Model file for the job. Use its own axes, mm. A direction names the side the tool comes from. Round coordinates to 2 decimals unless told otherwise and drop trailing zeros. Write each loop counter-clockwise with the first axis right and the second up, starting at its lowest first coordinate (ties: lowest second). Pieces come first, ordered by that corner, then holes. Notation, with made-up numbers: (9, 56) - (60, 56) arc R23 ccw to (60, 90) - close; hole circle Ø6 at (16.25, 84). An arc over 180 degrees is marked (long way). Answer as a JSON object with one key per item and string values. Group by question number.
from build123d import *

# Parameters (mm, degrees)
BOSS_EXTRUDE_1_DEPTH   = 4
BOSS_EXTRUDE_2_DEPTH   = 4
FILLET_1_R             = 5
SKETCH_6_W             = 24
SKETCH_6_H             = 30
BOSS_EXTRUDE_3_DEPTH   = 3.5
SKETCH_3_R             = 2.25
CUT_EXTRUDE_1_DEPTH    = 191.738695602
LINEAR_PATTERN_1_COUNT = 3
LINEAR_PATTERN_1_PITCH = 10
SKETCH_7_W             = 63.778369094
SKETCH_7_H             = 56.242484603
CUT_EXTRUDE_2_DEPTH    = 10
CHAMFER_3_SIZE         = 1
SKETCH_8_W             = 4.5
SKETCH_8_H             = 30
BOSS_EXTRUDE_4_DEPTH   = 3.5
CUT_EXTRUDE_START      = -10
CUT_EXTRUDE_3_DEPTH    = 10
F_4_0_4_HOLE_1_D       = 4
LINEAR_PATTERN_2_COUNT = 2
LINEAR_PATTERN_2_PITCH = 20


with BuildPart() as part:
    # Sketch 1 → Boss-Extrude 1 (new body)
    with BuildSketch(Plane.XZ.offset(2)):
        with BuildLine():
            Line((-59, 15), (-69, 15))
            Line((-69, 15), (-70, 15))
            Line((-70, 15), (-70, -15))
            Line((-70, -15), (-69, -15))
            Line((-69, -15), (69, -15))
            Line((69, -15), (70, -14))
            Line((70, -14), (70, -1))
            Line((70, -1), (69, 0))
            Line((69, 0), (-53, 0))
            ThreePointArc((-53, 0), (-56.535533906, 1.464466094), (-58, 5))
            Line((-58, 5), (-58, 15))
            Line((-58, 15), (-59, 15))
        make_face()
    extrude(amount=-BOSS_EXTRUDE_1_DEPTH)

    # Sketch 2 → Boss-Extrude 2 (add)
    with BuildSketch(Plane(origin=(0, 2, 0), x_dir=(1, 0, 0), z_dir=(0, 1, 0))):
        Polygon((-70, 15), (-190, 15), (-190, 0), (-82, 0), (-82, -15), (-70, -15), align=None)
    extrude(amount=-BOSS_EXTRUDE_2_DEPTH)

    # Fillet 1
    fillet_1_edges = [part.edges().sort_by_distance(p)[0] for p in [
        (-82, 0, 0),
    ]]
    fillet(fillet_1_edges, radius=FILLET_1_R)

    # Sketch 6 → Boss-Extrude 3 (add)
    with BuildSketch(Plane.XZ.offset(2)):
        with Locations((-70, 0)):
            Rectangle(SKETCH_6_W, SKETCH_6_H)
    extrude(amount=BOSS_EXTRUDE_3_DEPTH)

    # Sketch 3 → Cut-Extrude 1 (cut, through all)
    with BuildSketch(Plane(origin=(0, 2, 0), x_dir=(1, 0, 0), z_dir=(0, 1, 0))):
        with Locations(Location((-70, -10, 0), (0, 0, 270))):
            Circle(SKETCH_3_R)
    cut_extrude_1 = extrude(amount=-CUT_EXTRUDE_1_DEPTH, mode=Mode.SUBTRACT)

    # Linear Pattern 1: Cut-Extrude 1 ×3
    with Locations(*[(0, 0, -i * LINEAR_PATTERN_1_PITCH) for i in range(1, LINEAR_PATTERN_1_COUNT)]):
        add(cut_extrude_1, mode=Mode.SUBTRACT)

    # Sketch 7 → Cut-Extrude 2 (cut)
    with BuildSketch(Plane(origin=(0, 2, 0), x_dir=(1, 0, 0), z_dir=(0, 1, 0))):
        with Locations((81.889184547, 6.971733155)):
            Rectangle(SKETCH_7_W, SKETCH_7_H)
    extrude(amount=-CUT_EXTRUDE_2_DEPTH, mode=Mode.SUBTRACT)

    # Chamfer 3
    chamfer_3_edges = [part.edges().sort_by_distance(p)[0] for p in [
        (50, 0, -15),
        (50, 0, 0),
        (-190, 0, -15),
        (-190, 0, 0),
    ]]
    chamfer(chamfer_3_edges, length=CHAMFER_3_SIZE)

    # Sketch 8 → Boss-Extrude 4 (add)
    with BuildSketch(Plane.XZ.offset(5.5)):
        with Locations((-55.75, 0)):
            Rectangle(SKETCH_8_W, SKETCH_8_H)
        with Locations((-84.25, 0)):
            Rectangle(SKETCH_8_W, SKETCH_8_H)
    extrude(amount=-BOSS_EXTRUDE_4_DEPTH)

    # Sketch 9 → Cut-Extrude 3 (cut)
    with BuildSketch(Plane(origin=(0, -2, 0), x_dir=(1, 0, 0), z_dir=(0, 1, 0)).offset(CUT_EXTRUDE_START)):
        with BuildLine():
            Line((-53.5, -15), (-58, -15))
            Line((-58, -15), (-58, -5))
            ThreePointArc((-58, -5), (-56.708099244, -1.645898034), (-53.5, -0.025062814))
            Line((-53.5, -0.025062814), (-53.5, -15))
        make_face()
        with BuildLine():
            Line((-82, -15), (-86.5, -15))
            Line((-86.5, -15), (-86.5, -0.025062814))
            ThreePointArc((-86.5, -0.025062814), (-83.291900756, -1.645898034), (-82, -5))
            Line((-82, -5), (-82, -15))
        make_face()
    extrude(amount=CUT_EXTRUDE_3_DEPTH, mode=Mode.SUBTRACT)

    # Ø4.0 (4) Hole 1 (through all)
    with Locations(Plane(origin=(0, 2, 0), x_dir=(-1, 0, 0), z_dir=(0, 1, 0))):
        with Locations((60, -7.5)):
            f_4_0_4_hole_1 = Hole(F_4_0_4_HOLE_1_D / 2)

    # Linear Pattern 2: Ø4.0 (4) Hole 1 ×2
    with Locations(*[(-i * LINEAR_PATTERN_2_PITCH, 0, 0) for i in range(1, LINEAR_PATTERN_2_COUNT)]):
        add(f_4_0_4_hole_1, mode=Mode.SUBTRACT)


solid = part.part
(1) Slice it at D-D (x = -31). Write the cut outline in (y, z).
(2) Slice it at C-C (z = 10). Write the cut outline in (x, y).
(3) Drill centre lines: line 1 (X direction, y = -1.5, z = 10); line 2 (Z direction, x = -60, y = -3.5); line 3 (X direction, y = -4, z = -10). Where is each one in solid material? Low to high. Write a range as from..to.
(4) Slice it at A-A (x = -80). Write the cut outline in (y, z), then the cut area to 3 significant figures.
(5) 3-axis set-ups, long thin cutter, end or side, ignore diameter. For faces 4 (the flat face through (-139, 0, 0)), 5 (the flat face through (-58, -2, 10)), 6 (the flat face through (-2, -2, -8)), 7 (the cylindrical face through (-72.196, -1.697, -10.488)), 8 (the flat face through (-139, -2, -8)): which of +Z, -Z, +X, -X, +Y, -Y reach the whole face in a straight line?
(6) Pull direction Z, two halves, no side cores. Call faces 1 (the flat face through (-70, -2, 15)), 2 (the flat face through (-190, 0, -8)), 3 (the cylindrical face through (-72.196, -1.697, -0.488)): pulls with the +Z half, pulls with the -Z half, needs draft (parallel to the pull), parting line crosses it, or undercut.
(7) Slice it at B-B (y = 0.75). Write the cut outline in (x, z).
(8) Flat gauge pins, fed straight in: pin 1 (1 mm diameter, centred on y = -3.5, z = -5, fed in from +X); pin 2 (6.5 mm diameter, centred on x = -60, z = -7.5, fed in from +Y); pin 3 (4 mm diameter, centred on y = -3, z = 10, fed in from +X); pin 4 (1.5 mm diameter, centred on x = -139.5, y = -4.5, fed in from -Z). Where does each tip first touch, or does it go through?
Answer:
{
 "1": {"outline": "(-2, -15) - (2, -15) - (2, 0) - (-2, 0) - close"},
 "2": {"outline": "(-82, -5.5) - (-72.25, -5.5) - (-72.25, 2) - (-82, 2) - close; (-67.75, -5.5) - (-58, -5.5) - (-58, 2) - (-67.75, 2) - close"},
 "3": {"line 1": "-82..-72.25, -67.75..-58", "line 2": "-15..-9.5, -5.5..15", "line 3": "-86.5..-72.25, -67.75..-53.5"},
 "4": {"outline": "(-5.5, -15) - (2, -15) - (2, -9.5) - (-5.5, -9.5) - close; (-5.5, -5.5) - (2, -5.5) - (2, 15) - (-5.5, 15) - close", "area": "195 mm²"},
 "5": {"face 4": "+Z, -X, +Y, -Y", "face 5": "+Z, +X, +Y, -Y", "face 6": "+Z, -Z, +X, -Y", "face 7": "+Y, -Y", "face 8": "+Z, -Z, -X, -Y"},
 "6": {"face 1": "pulls with the +Z half", "face 2": "needs draft", "face 3": "undercut"},
 "7": {"outline": "(-190, -14) - (-189, -15) - (49, -15) - (50, -14) - (50, -1) - (49, 0) - (-53, 0) arc R5 cw to (-58, 5) - (-58, 15) - (-82, 15) - (-82, 5) arc R5 cw to (-87, 0) - (-189, 0) - (-190, -1) - close; hole circle Ø4 at (-80, -7.5); hole circle Ø4.5 at (-70, -10); hole circle Ø4.5 at (-70, 0); hole circle Ø4.5 at (-70, 10); hole circle Ø4 at (-60, -7.5)"},
 "8": {"pin 1": "x = -53.5", "pin 2": "y = 2", "pin 3": "x = -58", "pin 4": "through"}
}
